The listing builds one solid part. Answer for the finished solid, in the listing's coordinates (mm). Coordinates: 2 decimals unless noted, no trailing zeros. Order: outer loops, then holes, each group sorted by start corner. A loop starts at its lowest first (then second) coordinate and runs counter-clockwise, first axis right, second up. Notation, with made-up numbers: (3.5, 42) -> (50.5, 42) arc R19 ccw to (50.5, 73) -> close; hole circle Ø8 at (14, 86). An arc over 180 degrees is marked (long way). Return JSON: item names as keys, results as strings.
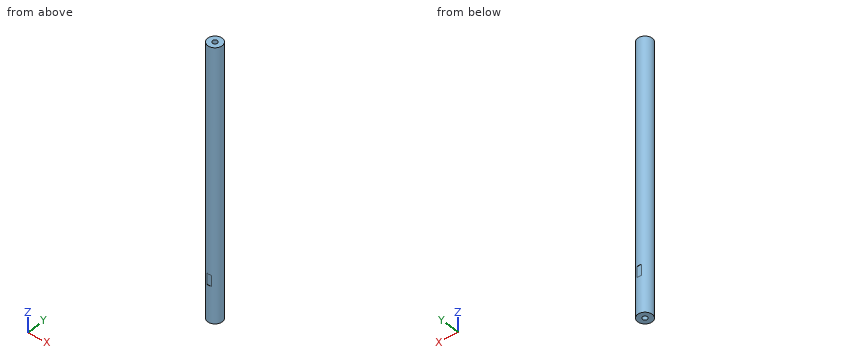
from build123d import *

# Parameters (mm, degrees)
SKETCH1_R             = 10
BOSS_EXTRUDE1_DEPTH   = 186
CUT_EXTRUDE1_START    = -65
CUT_EXTRUDE1_DEPTH    = 15
M8_TAPPED_HOLE1_D     = 6.8
M8_TAPPED_HOLE1_DEPTH = 19.75
M8_TAPPED_HOLE1_TIP   = 2.042926105
M8_TAPPED_HOLE2_D     = 6.8
M8_TAPPED_HOLE2_DEPTH = 19.75
M8_TAPPED_HOLE2_TIP   = 2.042926105


with BuildPart() as part:
    # Sketch1 → Boss-Extrude1 (new, symmetric)
    with BuildSketch(Plane.XY):
        with Locations(Location((0, 0, 0), (0, 0, 180))):
            Circle(SKETCH1_R)
    extrude(amount=BOSS_EXTRUDE1_DEPTH, both=True)

    # Sketch2 → Cut-Extrude1 (cut)
    with BuildSketch(Plane(origin=(0, 0, -186), x_dir=(-1, 0, 0), z_dir=(0, 0, -1)).offset(CUT_EXTRUDE1_START)):
        with BuildLine():
            Line((-3.122498999, -9.5), (3.122498999, -9.5))
            ThreePointArc((3.122498999, -9.5), (0, -10), (-3.122498999, -9.5))
        make_face()
        with BuildLine():
            Line((-3.122498999, 9.5), (3.122498999, 9.5))
            ThreePointArc((3.122498999, 9.5), (0, 10), (-3.122498999, 9.5))
        make_face()
    extrude(amount=CUT_EXTRUDE1_DEPTH, mode=Mode.SUBTRACT)

    # M8 Tapped Hole1
    with Locations(Plane(origin=(0, 0, -186), x_dir=(-1, 0, 0), z_dir=(0, 0, -1))):
        with Locations((0, 0)):
            Hole(M8_TAPPED_HOLE1_D / 2, depth=M8_TAPPED_HOLE1_DEPTH)
            with Locations((0, 0, -(M8_TAPPED_HOLE1_DEPTH + M8_TAPPED_HOLE1_TIP / 2))):  # 118° drill point
                Cone(0, M8_TAPPED_HOLE1_D / 2, M8_TAPPED_HOLE1_TIP, mode=Mode.SUBTRACT)

    # M8 Tapped Hole2
    with Locations(Plane.XY.offset(186)):
        with Locations((0, 0)):
            Hole(M8_TAPPED_HOLE2_D / 2, depth=M8_TAPPED_HOLE2_DEPTH)
            with Locations((0, 0, -(M8_TAPPED_HOLE2_DEPTH + M8_TAPPED_HOLE2_TIP / 2))):  # 118° drill point
                Cone(0, M8_TAPPED_HOLE2_D / 2, M8_TAPPED_HOLE2_TIP, mode=Mode.SUBTRACT)


solid = part.part
1. The part is cut by section A-A on z = 92. Give the vertices of the cut face in (x, y).
Answer block:
{"outline": "circle Ø20 at (0, 0)"}
2. Consider line 1 (Y direction, x = 0, z = -173.75); line 2 (Y direction, x = 0.25, z = -50); line 3 (Y direction, x = -1, z = 121). Determine where each line is inside the solid, lowest interval first. Write a range as from..to.
Answer block:
{"line 1": "y = -10..-3.4, 3.4..10", "line 2": "y = -10..10", "line 3": "y = -9.95..9.95"}
3. Each of these flat-tipped pins is pushed along its axis until it touches: pin 1 Ø5 at (y, z) = (-6, -71) entering from +X; pin 2 Ø5 at (x, z) = (1, 135) entering from -Y; pin 3 Ø4 at (x, y) = (0, 0) entering from +Z; pin 4 Ø3 at (x, z) = (1, -127.5) entering from +Y. Where does it stop, or does it pass through?
Answer block:
{"pin 1": "stops at x = 9.37", "pin 2": "stops at y = -10", "pin 3": "stops at z = 165.41", "pin 4": "stops at y = 9.5"}
